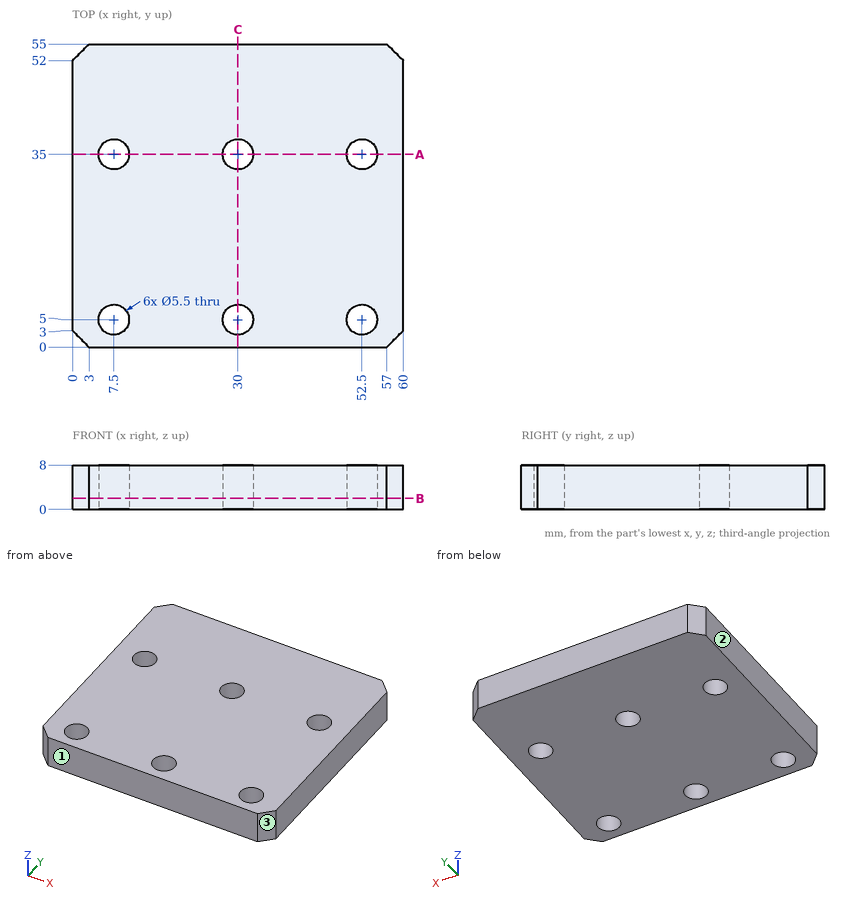
Check sheet for the drawn part. Datum: minimum x, y, z corner. Units: mm. Round coordinates to 2 decimals unless told otherwise and drop trailing zeros. Order: outer loops, then holes, each group sorted by start corner. A loop starts at its lowest first (then second) coordinate and runs counter-clockwise, first axis right, second up.
(1) Cross-section at A-A, the plane y = 35. Enter the section's corners in (x, z), and give its area (3 significant figures).
(2) Draft check along X on the marked faces 1, 2 and 3. Enter one of: pulls with the +X half, pulls with the -X half, needs draft (parallel to the pull), parting line crosses it, or undercut.
(3) Scan lines: probe 1 along Y at (x, z) = (52.5, 4.25); probe 2 along X at (y, z) = (3, 7.5); probe 3 along X at (y, z) = (6, 1.5). Record each from-to range of solid material in increasing order.
(4) Cross-section at B-B, the plane z = 2. Enter the section's corners in (x, y).
(5) Cross-section at C-C, the plane x = 30. Enter the section's corners in (y, z).
(6) Go/stop test with a flat-tipped pin: P1, Ø6.5, axis at x = 30, y = 35, coming from the +Z side. Record where the tip stops, or that it passes through.
Check sheet entries:
1. outline: (0, 0) - (4.75, 0) - (4.75, 8) - (0, 8) - close; (10.25, 0) - (27.25, 0) - (27.25, 8) - (10.25, 8) - close; (32.75, 0) - (49.75, 0) - (49.75, 8) - (32.75, 8) - close; (55.25, 0) - (60, 0) - (60, 8) - (55.25, 8) - close
1. area: 348 mm2
2. face 1: needs draft
2. face 2: pulls with the -X half
2. face 3: pulls with the +X half
3. probe 1: y = 0 to 2.25, 7.75 to 32.25, 37.75 to 55
3. probe 2: x = 0 to 5.61, 9.39 to 28.11, 31.89 to 50.61, 54.39 to 60
3. probe 3: x = 0 to 4.94, 10.06 to 27.44, 32.56 to 49.94, 55.06 to 60
4. outline: (0, 3) - (3, 0) - (57, 0) - (60, 3) - (60, 52) - (57, 55) - (3, 55) - (0, 52) - close; hole circle Ø5.5 at (7.5, 5); hole circle Ø5.5 at (7.5, 35); hole circle Ø5.5 at (30, 5); hole circle Ø5.5 at (30, 35); hole circle Ø5.5 at (52.5, 5); hole circle Ø5.5 at (52.5, 35)
5. outline: (0, 0) - (2.25, 0) - (2.25, 8) - (0, 8) - close; (7.75, 0) - (32.25, 0) - (32.25, 8) - (7.75, 8) - close; (37.75, 0) - (55, 0) - (55, 8) - (37.75, 8) - close
6. P1: stops at z = 8
